The drawing under review shows one solid part. Ordinate dimensions are in mm from its lowest x, y, z. Coordinates: 2 decimals unless noted, no trailing zeros. Write each loop counter-clockwise with the first axis right and the second up, starting at its lowest first coordinate (ties: lowest second). Pieces come first, ordered by that corner, then holes.
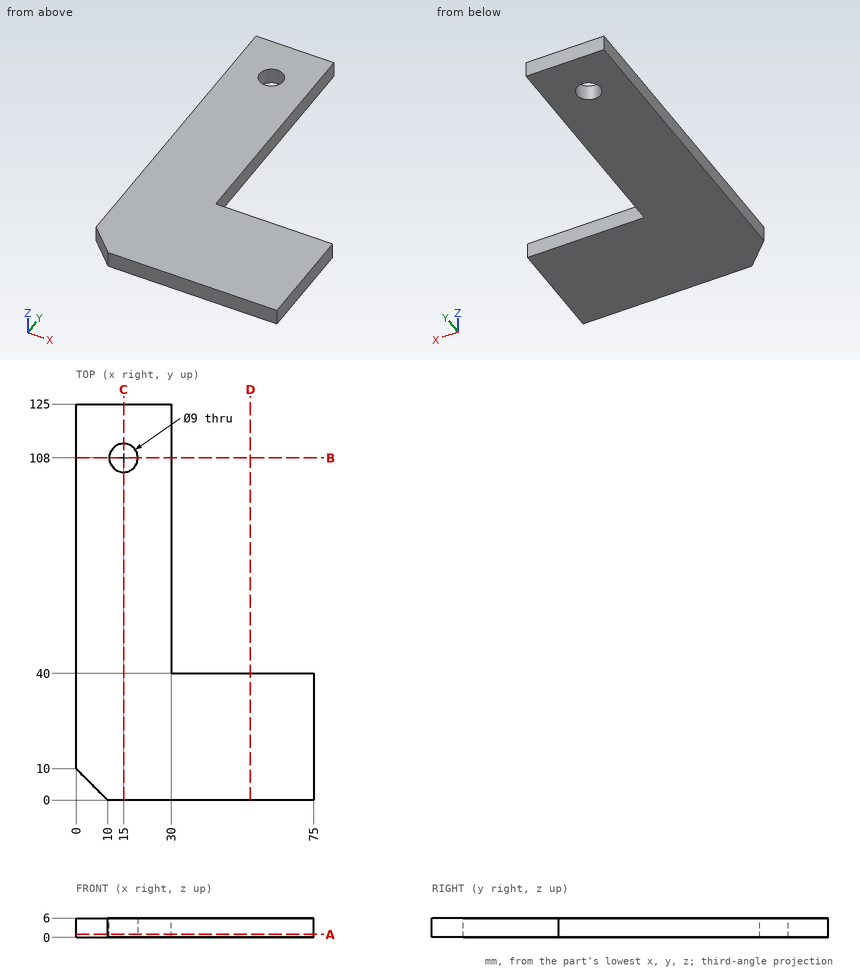
Q1. Add section A-A (z = 0.95). State the section outline as (x, y) points.
Ans:
outline: (0, 10) - (10, 0) - (75, 0) - (75, 40) - (30, 40) - (30, 125) - (0, 125) - close; hole circle Ø9 at (15, 108)
Q2. For probe 1 along Y at (x, z) = (15, 3.5); probe 2 along X at (y, z) = (90.5, 4.9); probe 3 along Y at (x, z) = (18.5, 3.25), list the stretches that pass through material, from the lowest coordinate up.
Ans:
probe 1: y = 0 to 103.5, 112.5 to 125
probe 2: x = 0 to 30
probe 3: y = 0 to 105.17, 110.83 to 125
Q3. Add section B-B (y = 108). State the section outline as (x, z) points, then the cut area to 3 significant figures.
Ans:
outline: (0, 0) - (10.5, 0) - (10.5, 6) - (0, 6) - close; (19.5, 0) - (30, 0) - (30, 6) - (19.5, 6) - close
area: 126 mm2
Q4. Add section D-D (x = 55). State the section outline as (y, z) points.
Ans:
outline: (0, 0) - (40, 0) - (40, 6) - (0, 6) - close
Q5. Add section C-C (x = 15). State the section outline as (y, z) points, then the cut area to 3 significant figures.
Ans:
outline: (0, 0) - (103.5, 0) - (103.5, 6) - (0, 6) - close; (112.5, 0) - (125, 0) - (125, 6) - (112.5, 6) - close
area: 696 mm2
Q6. Clearance check with a flat-ended pin moving along its axis: pin 1 Ø1.8 at (y, z) = (77, 1.5) entering from +X. State where the tip first meets the part, or that it passes through.
Ans:
pin 1: stops at x = 30
